```python
from build123d import *

# Parameters (mm, degrees)
SKETCH2_R               = 0.3
SKETCH4_W               = 1
SKETCH4_H               = 1
BOSS_EXTRUDE1_DEPTH     = 3
CUT_EXTRUDE1_DEPTH      = 23.185130234
CUT_EXTRUDE1_DEPTH_BACK = 23.185130234


with BuildPart() as part:
    # Sweep1: sweep along a curve in space
    with BuildLine() as sweep1_path:
        Line((0, 0, 0), (0, 12.1, 0))
        ThreePointArc((0, 12.1, 0), (0.117157288, 12.382842712, 0), (0.4, 12.5, 0))
        Line((0.4, 12.5, 0), (2.4, 12.5, 0))
        ThreePointArc((2.4, 12.5, 0), (3.814213562, 12.5, -0.585786438), (4.4, 12.5, -2))
        Line((4.4, 12.5, -2), (4.4, 12.5, -15))
        ThreePointArc((4.4, 12.5, -15), (3.814213562, 12.5, -16.414213562), (2.4, 12.5, -17))
        Line((2.4, 12.5, -17), (0.4, 12.5, -17))
        ThreePointArc((0.4, 12.5, -17), (0.117157288, 12.382842712, -17), (0, 12.1, -17))
        Line((0, 12.1, -17), (0, 0, -17))
    # Sketch2 → Sweep1 (sweep)
    with BuildSketch(Plane(origin=(0, 0, 0), x_dir=(1, 0, 0), z_dir=(0, 1, 0))):
        Circle(SKETCH2_R)
    sweep(path=sweep1_path.line)

    # Sketch4 → Boss-Extrude1 (add)
    with BuildSketch(Plane(origin=(0, 0, 0), x_dir=(-1, 0, 0), z_dir=(0, -1, 0))):
        with Locations((0, 17)):
            Rectangle(SKETCH4_W, SKETCH4_H)
        Rectangle(SKETCH4_W, SKETCH4_H)
    extrude(amount=-BOSS_EXTRUDE1_DEPTH)

    # Sketch5 → Cut-Extrude1 (cut, two sides: drawn at the far end of the back side and taken through both)
    with BuildSketch(Plane(origin=(0, 0, 0), x_dir=(0, 0, -1), z_dir=(1, 0, 0)).offset(-CUT_EXTRUDE1_DEPTH_BACK)):
        Polygon((-0.5, 0), (1.563257824, 2.946637548), (15.436742176, 2.946637548), (17.5, 0), align=None)
    extrude(amount=CUT_EXTRUDE1_DEPTH + CUT_EXTRUDE1_DEPTH_BACK, mode=Mode.SUBTRACT)


solid = part.part
```
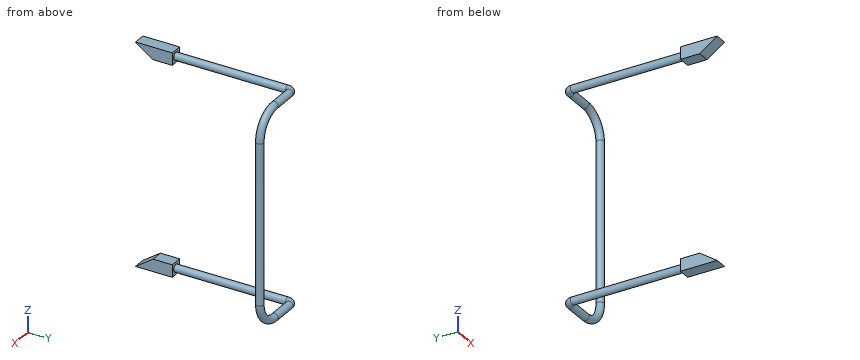
Verification items for the finished model (mm, model axes). Coordinates: 2 decimals unless noted, no trailing zeros. Write each loop counter-clockwise with the first axis right and the second up, starting at its lowest first coordinate (ties: lowest second). Pieces come first, ordered by that corner, then holes. Notation, with made-up numbers: M 50,49 L 100,49 A31 cw 100,87 Z; hole C 89,-35 d11. An arc over 180 degrees is marked long. One line per item, written item: value.
Item 1: Gauge pin test, flat ends, axial feed: pin 1 Ø2 at (x, z) = (1.5, -9) entering from -Y; pin 2 Ø2 at (x, y) = (1, 3) entering from -Z; pin 3 Ø0.5 at (x, z) = (0, -17) entering from +Y; pin 4 Ø0.5 at (y, z) = (1.5, 0) entering from +X. Record the tip position at first contact, or that the pin passes through.
Check sheet entries:
pin 1: passes through
pin 2: stops at z = -17.5
pin 3: stops at y = 12.78
pin 4: stops at x = 0.5
Item 2: Section check C-C, the plane y = 1. Record the boundary of the cut face in (x, z).
Check sheet entries:
outline: M -0.5,-17.5 L 0.5,-17.5 L 0.5,-16.8 L -0.5,-16.8 Z; M -0.5,-0.2 L 0.5,-0.2 L 0.5,0.5 L -0.5,0.5 Z
Item 3: Section check D-D, the plane z = -11. Record the boundary of the cut face in (x, y), plus the area to 3 significant figures.
Check sheet entries:
outline: C 4.4,12.5 d0.6
area: 0.283 mm^2
Item 4: Section check B-B, the plane x = 0.75. Record the boundary of the cut face in (y, z), plus the area to 3 significant figures.
Check sheet entries:
outline: C 12.5,-17 d0.6; C 12.5,0 d0.6
area: 0.565 mm^2
Item 5: Section check A-A, the plane y = 2.5. Record the boundary of the cut face in (x, z).
Check sheet entries:
outline: M -0.5,-17.5 L 0.5,-17.5 L 0.5,-16.5 L -0.5,-16.5 Z; M -0.5,-0.5 L 0.5,-0.5 L 0.5,0.5 L -0.5,0.5 Z
Item 6: Scan lines: line 1 along Z through (x, y) = (0.45, 2.25); line 2 along Z through (x, y) = (0.1, 1.25); line 3 along Y through (x, z) = (4, -1). Record each from-to range of solid material in increasing order.
Check sheet entries:
line 1: z = -17.5 to -16.5, -0.5 to 0.5
line 2: z = -17.5 to -16.62, -0.38 to 0.5
line 3: y = 12.22 to 12.78
